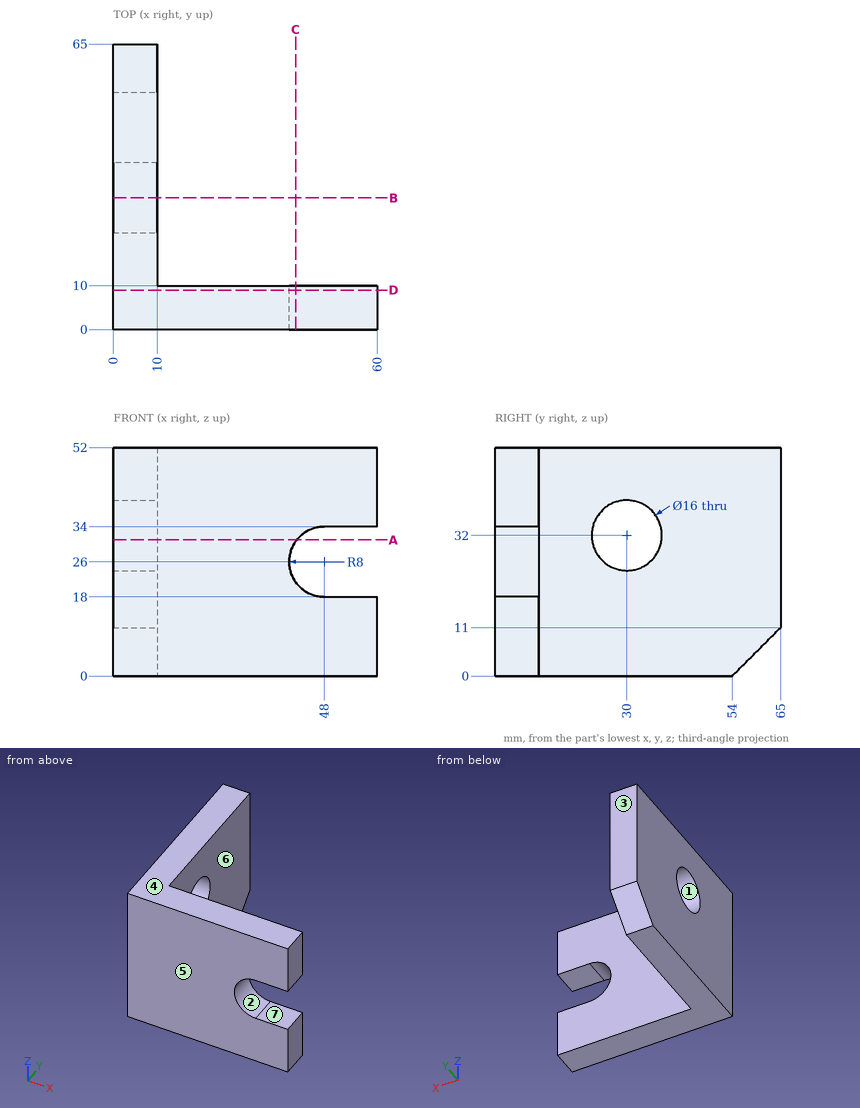
Can you work these out from the drawing? Everything is in mm from the part's minimum corner. A direction names the side the tool comes from. Coordinates: 2 decimals unless noted, no trailing zeros. Write each loop counter-clockwise with the first axis right and the second up, starting at its lowest first coordinate (ties: lowest second). Pieces come first, ordered by that corner, then holes. Notation, with made-up numbers: (-16, 63.25) -> (-4, 63.25) arc R26 ccw to (-4, 100.25) -> close; hole circle Ø3 at (54, -12.75). An arc over 180 degrees is marked (long way). Write each question's results on one line, items separated by ' | '. Start each with the question number.
Q1. We'd pull the mould along Z, two halves only. Please class the marked faces 1, 2, 3 and 4: +Z half, -Z half, draft (parallel to the pull), parting line (faces both ways), or undercut.
Q2. Imagine slicing it at D-D (y = 9). Write out the boundary of the cut face in (x, z).
Q3. Imagine slicing it at C-C (x = 41.5). Write out the boundary of the cut face in (y, z).
Q4. Imagine slicing it at B-B (y = 30). Write out the boundary of the cut face in (x, z).
Q5. On a 3-axis mill with a long thin cutter (end or side, diameter ignored), from which of +Z, -Z, +X, -X, +Y, -Y can I reach the whole of each face in a straight line? I mean the marked faces 5, 6 and 7. Say none if no direction works.
Q6. Imagine slicing it at A-A (z = 31). Write out the boundary of the cut face in (x, y) (3 decimals).
Q7. If I drill on probe 1 along Z at (x, y) = (5, 30); probe 2 along X at (y, z) = (62, 35), over which ranges is the centre line in solid material (lowest first)?
Taken from the geometry:
1) face 1: undercut | face 2: undercut | face 3: draft | face 4: +Z half
2) outline: (0, 0) -> (60, 0) -> (60, 18) -> (48, 18) arc R8 cw to (48, 34) -> (60, 34) -> (60, 52) -> (0, 52) -> close
3) outline: (0, 0) -> (10, 0) -> (10, 21.34) -> (0, 21.34) -> close; (0, 30.66) -> (10, 30.66) -> (10, 52) -> (0, 52) -> close
4) outline: (0, 0) -> (10, 0) -> (10, 24) -> (0, 24) -> close; (0, 40) -> (10, 40) -> (10, 52) -> (0, 52) -> close
5) face 5: +Z, -Z, +X, -X, -Y | face 6: +Z, -Z, +X, +Y | face 7: +X, +Y, -Y
6) outline: (0, 0) -> (41.755, 0) -> (41.755, 10) -> (10, 10) -> (10, 22.063) -> (0, 22.063) -> close; (0, 37.937) -> (10, 37.937) -> (10, 65) -> (0, 65) -> close
7) probe 1: z = 0 to 24, 40 to 52 | probe 2: x = 0 to 10
